Verification items for the finished model (mm, model axes). Face numbers are marked on the shaded views. A direction names the side the tool comes from. Give positions to 0.01 mm unless a question says otherwise; leave off trailing zeros. Loops run counter-clockwise (first coordinate to the right, second up) from the corner with the lowest first, then second, coordinate; pieces in that order, holes last. Notation, with made-up numbers: M -37.5,70 L 10.5,70 A21 ccw 10.5,91 Z; hole C 56.5,29 d3. An arc over 180 degrees is marked long. Use a Markdown table: item, result.
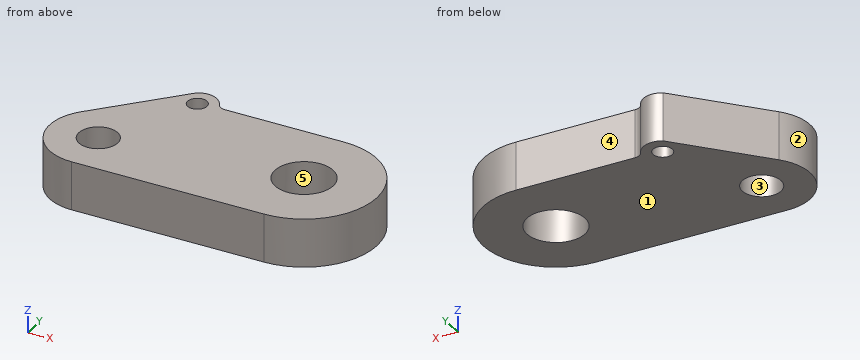
from build123d import *

# Parameters (mm, degrees)
SKETCH1_R           = 3
SKETCH1_R_2         = 1
SKETCH1_R_3         = 2
BOSS_EXTRUDE1_DEPTH = 5


with BuildPart() as part:
    # Sketch1 → Boss-Extrude1 (new body)
    with BuildSketch(Plane.XY):
        with BuildLine():
            Line((-19.84, -7.5), (0, -7.5))
            ThreePointArc((0, -7.5), (7.5, 0), (0, 7.5))
            Line((0, 7.5), (-12.252821971, 7.5))
            ThreePointArc((-12.252821971, 7.5), (-12.792883696, 7.658374588), (-13.161881314, 8.083333333))
            ThreePointArc((-13.161881314, 8.083333333), (-14.360041425, 9.15148662), (-15.957538412, 8.994826253))
            Line((-15.957538412, 8.994826253), (-23.496768508, 0.9099918))
            ThreePointArc((-23.496768508, 0.9099918), (-24.425300372, -4.493745345), (-19.84, -7.5))
        make_face()
        Circle(SKETCH1_R, mode=Mode.SUBTRACT)
        with Locations((-14.98, 7.25)):
            Circle(SKETCH1_R_2, mode=Mode.SUBTRACT)
        with Locations((-19.84, -2.5)):
            Circle(SKETCH1_R_3, mode=Mode.SUBTRACT)
    extrude(amount=BOSS_EXTRUDE1_DEPTH)


solid = part.part
(1) Draft check along Y on the marked faces 1, 2 and 3. Enter one of: +Y half, -Y half, draft (parallel to the pull), parting line (faces both ways), or undercut.
Results below:
| item | result |
|---|---|
| face 1 | draft |
| face 2 | parting line |
| face 3 | undercut |
(2) Cross-section at A-A on z = 2.6. Record the cut outline in (x, y).
Results below:
| item | result |
|---|---|
| outline | M -23.5,0.91 A5 ccw -19.84,-7.5 L 0,-7.5 A7.5 ccw 0,7.5 L -12.25,7.5 A1 cw -13.16,8.08 A2 ccw -15.96,8.99 Z; hole C -19.84,-2.5 d4; hole C -14.98,7.25 d2; hole C 0,0 d6 |
(3) Gauge pin test, flat ends, axial feed: P1, Ø3, axis at x = -14.98, y = 7.25, coming from the -Z side; P2, Ø3.5, axis at x = -19.84, y = -2.5, coming from the +Z side. Record the tip position at first contact, or that the pin passes through.
Results below:
| item | result |
|---|---|
| P1 | z = 0 |
| P2 | through |
(4) Set-up check for the marked faces 4 and 5: record each of +Z, -Z, +X, -X, +Y, -Y from which the full face is reachable in a straight line by a thin tool's end or side.
Results below:
| item | result |
|---|---|
| face 4 | +Z, -Z, +X, +Y |
| face 5 | +Z, -Z |
(5) Cross-section at C-C on y = 2.5. Record the cut outline in (x, z), then the cut area to 3 significant figures.
Results below:
| item | result |
|---|---|
| outline | M -22.01,0 L -1.66,0 L -1.66,5 L -22.01,5 Z; M 1.66,0 L 7.07,0 L 7.07,5 L 1.66,5 Z |
| area | 129 mm^2 |
(6) Material ranges on line 1 (X direction, y = -1.75, z = 1.65); line 2 (Y direction, x = -18, z = 4.5); line 3 (Y direction, x = -19.84, z = 2.35), recorded low to high.
Results below:
| item | result |
|---|---|
| line 1 | -24.78 to -21.69, -17.99 to -2.44, 2.44 to 7.29 |
| line 2 | -7.5 to -3.28, -1.72 to 6.8 |
| line 3 | -7.5 to -4.5, -0.5 to 4.83 |
(7) Cross-section at B-B on x = -14.98. Record the cut outline in (y, z), then the cut area to 4 significant figures.
Results below:
| item | result |
|---|---|
| outline | M -7.5,0 L 6.25,0 L 6.25,5 L -7.5,5 Z; M 8.25,0 L 9.25,0 L 9.25,5 L 8.25,5 Z |
| area | 73.75 mm^2 |
(8) Cross-section at D-D on x = -10. Record the cut outline in (y, z), then the cut area to 3 significant figures.
Results below:
| item | result |
|---|---|
| outline | M -7.5,0 L 7.5,0 L 7.5,5 L -7.5,5 Z |
| area | 75.0 mm^2 |
